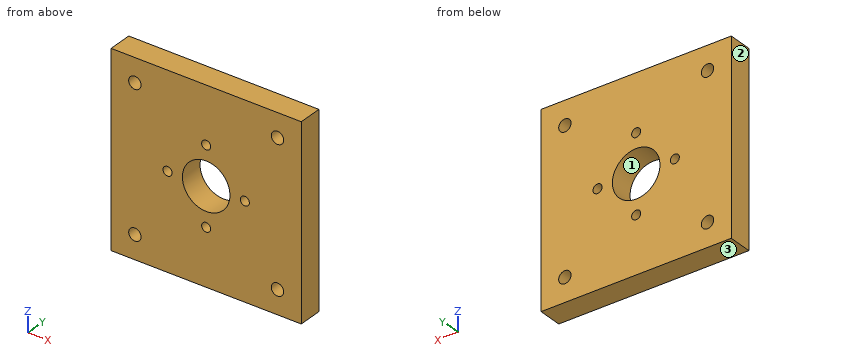
```python
from build123d import *

# Parameters (mm, degrees)
BASE_PLATE_PROFILE_W        = 400
BASE_PLATE_PROFILE_H        = 400
BASE_PLATE_PROFILE_R        = 50
BASE_PLATE_PROFILE_R_2      = 13
BASE_PLATE_PROFILE_R_3      = 9.5
BASE_PLATE_400X400X50_DEPTH = 25


with BuildPart() as part:
    # Base Plate Profile → Base Plate 400x400x50 (new, symmetric)
    with BuildSketch(Plane(origin=(0, 0, 0), x_dir=(1, 0, 0), z_dir=(0, 1, 0))):
        Rectangle(BASE_PLATE_PROFILE_W, BASE_PLATE_PROFILE_H)
        with Locations(Location((0, 0, 0), (0, 0, 270))):
            Circle(BASE_PLATE_PROFILE_R, mode=Mode.SUBTRACT)
        with Locations(Location((150, 150, 0), (0, 0, 270))):
            Circle(BASE_PLATE_PROFILE_R_2, mode=Mode.SUBTRACT)
        with Locations(Location((-150, 150, 0), (0, 0, 90))):
            Circle(BASE_PLATE_PROFILE_R_2, mode=Mode.SUBTRACT)
        with Locations(Location((150, -150, 0), (0, 0, 90))):
            Circle(BASE_PLATE_PROFILE_R_2, mode=Mode.SUBTRACT)
        with Locations(Location((-150, -150, 0), (0, 0, 270))):
            Circle(BASE_PLATE_PROFILE_R_2, mode=Mode.SUBTRACT)
        with Locations(Location((0, 81.3, 0), (0, 0, 270))):
            Circle(BASE_PLATE_PROFILE_R_3, mode=Mode.SUBTRACT)
        with Locations(Location((0, -81.3, 0), (0, 0, 90))):
            Circle(BASE_PLATE_PROFILE_R_3, mode=Mode.SUBTRACT)
        with Locations(Location((-81.3, 0, 0), (0, 0, 270))):
            Circle(BASE_PLATE_PROFILE_R_3, mode=Mode.SUBTRACT)
        with Locations(Location((81.3, 0, 0), (0, 0, 90))):
            Circle(BASE_PLATE_PROFILE_R_3, mode=Mode.SUBTRACT)
    extrude(amount=BASE_PLATE_400X400X50_DEPTH, both=True)


solid = part.part
```
Check sheet for the modelled part. Datum: model origin and axes. Units: mm. Face numbers are marked on the shaded views. Round coordinates to 2 decimals unless told otherwise and drop trailing zeros. Write each loop counter-clockwise with the first axis right and the second up, starting at its lowest first coordinate (ties: lowest second). Pieces come first, ordered by that corner, then holes. Notation, with made-up numbers: M 79,-31 L 122,-31 A24 cw 122,-7 Z; hole C 26.5,84.5 d1. An arc over 180 degrees is marked long. Write item = value, one per line. Start each with the question number.
1. Section check C-C, the plane x = 81.3. Record the cut outline in (y, z).
2. Section check A-A, the plane z = 0. Record the cut outline in (x, y).
3. Section check B-B, the plane y = 9. State how many separate pieces and enclosed holes the cut face has, then the cut area to 3 significant figures.
4. Gauge pin test, flat end, axial feed: pin 1 (15 mm diameter, centred on x = -81.3, z = 0, fed in from +Y). Record the tip position at first contact, or that the pin passes through.
5. Release check for a two-part mould opening along X. For the marked faces 1, 2 and 3 record: pulls with the +X half, pulls with the -X half, needs draft (parallel to the pull), parting line crosses it, or undercut.
6. Section check D-D, the plane z = 145.5. Record the cut outline in (x, y), then the cut area to 3 significant figures.
7. Scan lines: line 1 (Z direction, x = -149, y = -8); line 2 (X direction, y = 0.5, z = 81.3); line 3 (X direction, y = 0, z = 140.5). Record each from-to range of solid material in increasing order. Write a range as [from, to].
Results found:
q1.outline = M -25,-200 L 25,-200 L 25,-9.5 L -25,-9.5 Z; M -25,9.5 L 25,9.5 L 25,200 L -25,200 Z
q2.outline = M -200,-25 L -90.8,-25 L -90.8,25 L -200,25 Z; M -71.8,-25 L -50,-25 L -50,25 L -71.8,25 Z; M 50,-25 L 71.8,-25 L 71.8,25 L 50,25 Z; M 90.8,-25 L 200,-25 L 200,25 L 90.8,25 Z
q3.separate_pieces = 1
q3.enclosed_holes = 9
q3.area = 149,000 mm^2
q4.pin_1 = through
q5.face_1 = undercut
q5.face_2 = pulls with the -X half
q5.face_3 = needs draft
q6.outline = M -200,-25 L -162.2,-25 L -162.2,25 L -200,25 Z; M -137.8,-25 L 137.8,-25 L 137.8,25 L -137.8,25 Z; M 162.2,-25 L 200,-25 L 200,25 L 162.2,25 Z
q6.area = 17,600 mm^2
q7.line_1 = [-200, -162.96], [-137.04, 137.04], [162.96, 200]
q7.line_2 = [-200, -9.5], [9.5, 200]
q7.line_3 = [-200, -158.87], [-141.13, 141.13], [158.87, 200]
